```python
from build123d import *

# Parameters (mm, degrees)
CUT_EXTRUDE1_DEPTH = 1.833333333


with BuildPart() as part:
    # Sketch1 → Revolve1 (revolve)
    with BuildSketch(Plane.XY, mode=Mode.PRIVATE) as revolve1_sk:
        Polygon((-5.5, 0), (-5.5, 2.614834957), (-5.234834957, 2.88), (-4.75, 2.88), (-4.63, 3), (-0.87, 3), (-0.75, 2.88), (0, 2.88), (0, 1.5), (5.6935, 1.5), (6, 1.1935), (6, 0), align=None)
    revolve(revolve1_sk.sketch.rotate(Axis((6, 0, 0), (-1, 0, 0)), 270), axis=Axis((6, 0, 0), (-1, 0, 0)))

    # Sketch2 → Cut-Revolve1 (revolve, cut)
    with BuildSketch(Plane.XY, mode=Mode.PRIVATE) as cut_revolve1_sk:
        Polygon((-5.5, 0), (-5.5, 0.91), (-5.11, 0.52), (-3.05022214, 0.52), (-2.75, 0), align=None)
    revolve(cut_revolve1_sk.sketch.rotate(Axis((-2.75, 0, 0), (-1, 0, 0)), 270), axis=Axis((-2.75, 0, 0), (-1, 0, 0)), mode=Mode.SUBTRACT)

    # Sketch3 → Cut-Extrude1 (cut)
    with BuildSketch(Plane(origin=(-5.5, 0, 0), x_dir=(0, 0, -1), z_dir=(1, 0, 0))):
        Polygon((-0.65, 0.375277675), (-0.65, -0.375277675), (0, -0.75055535), (0.65, -0.375277675), (0.65, 0.375277675), (0, 0.75055535), align=None)
    extrude(amount=CUT_EXTRUDE1_DEPTH, mode=Mode.SUBTRACT)


solid = part.part
```
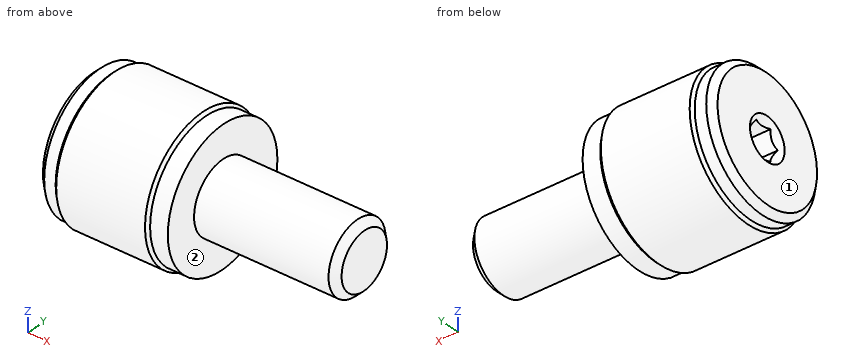
The model under review builds one solid part; all positions refer to its coordinate system, in mm. Face numbers are marked on the shaded views. A direction names the side the tool comes from. Coordinates: 2 decimals unless noted, no trailing zeros. Order: outer loops, then holes, each group sorted by start corner. A loop starts at its lowest first (then second) coordinate and runs counter-clockwise, first axis right, second up. Notation, with made-up numbers: M -28,77.25 L -23,77.25 A24 cw -23,111.25 Z; hole C -26,79.25 d5. An arc over 180 degrees is marked long. One line per question, with ' | ' between items.
(1) Add section C-C, the plane x = 2.5. Write out the cut boundary in (y, z), then the cut area to 3 significant figures.
Geometry results:
outline: C 0,0 d3 | area: 7.07 mm²
(2) Add section A-A, the plane x = -5. Write out the cut boundary in (y, z).
Geometry results:
outline: C 0,0 d5.76; hole M -0.75,0 L -0.38,-0.65 L 0.38,-0.65 L 0.75,0 L 0.38,0.65 L -0.38,0.65 Z
(3) Machinability: for the marked faces 1 and 2, which of the approach directions +Z, -Z, +X, -X, +Y, -Y give a long, thin tool a straight path to every point of the face, cutting with its end or side? Answer none if there is none.
Geometry results:
face 1: +Z, -Z, -X, +Y, -Y | face 2: +X
(4) Add section B-B, the plane x = -3.25. Write out the cut boundary in (y, z), then the cut area to 3 significant figures.
Geometry results:
outline: C 0,0 d6; hole C 0,0 d1.04 | area: 27.4 mm²
(5) Insertion check: pin 1 (2 mm diameter, centred on x = 4, y = 2, fed in from +Z); pin 2 (2 mm diameter, centred on x = 4, z = -0.5, fed in from +Y). Each pin has a flat end and moves straight along its axis. Give the tip position at first contact, or say it passes through.
Geometry results:
pin 1: stops at z = 1.12 | pin 2: stops at y = 1.5
(6) For probe 1 along Y at (x, z) = (-3.3, 0); probe 2 along X at (y, z) = (0.1, -2.2); probe 3 along Z at (x, y) = (3.5, 0.1), list the stretches that pass through material, from the lowest coordinate up. Write a range as from..to.
Geometry results:
probe 1: y = -3..-0.52, 0.52..3 | probe 2: x = -5.5..0 | probe 3: z = -1.5..1.5
